For this review, take the finished solid that the model builds, in its own axes (mm). A direction names the side the tool comes from. Coordinates: 2 decimals unless noted, no trailing zeros. Loops run counter-clockwise (first coordinate to the right, second up) from the corner with the lowest first, then second, coordinate; pieces in that order, holes last. Notation, with made-up numbers: M -32,48 L 26,48 A16 ccw 26,73 Z; hole C -25,21.25 d8. An arc over 180 degrees is marked long. Use one line per item in the form item = value.
```python
from build123d import *

# Parameters (mm, degrees)
SKETCH1_R             = 25.1
BOSS_EXTRUDE1_DEPTH   = 6
FILLET1_R             = 4
FILLET2_R             = 2
CHAMFER1_SIZE         = 1
M5_TAPPED_HOLE2_D     = 4.2
M5_TAPPED_HOLE1_D     = 4.2
M5_TAPPED_HOLE1_DEPTH = 14
M5_TAPPED_HOLE1_TIP   = 1.2618073
CHAMFER2_SIZE         = 1


with BuildPart() as part:
    # Sketch1 → Boss-Extrude1 (new, symmetric)
    with BuildSketch(Plane(origin=(0, 0, 0), x_dir=(0, 0, -1), z_dir=(1, 0, 0))):
        Polygon((-45, 0), (45, 0), (45, 12), (30, 12), (30, 72), (-30, 72), (-30, 12), (-45, 12), align=None)
        with Locations((0, 42)):
            Circle(SKETCH1_R, mode=Mode.SUBTRACT)
    extrude(amount=BOSS_EXTRUDE1_DEPTH, both=True)

    # Fillet1
    fillet1_edges = [part.edges().sort_by_distance(p)[0] for p in [
        (0, 72, 30),
        (0, 72, -30),
    ]]
    fillet(fillet1_edges, radius=FILLET1_R)

    # Fillet2
    fillet2_edges = [part.edges().sort_by_distance(p)[0] for p in [
        (0, 12, 30),
        (0, 12, -30),
    ]]
    fillet(fillet2_edges, radius=FILLET2_R)

    # Chamfer1
    chamfer1_edges = [part.edges().sort_by_distance(p)[0] for p in [
        (0, 12, 45),
        (0, 12, -45),
    ]]
    chamfer(chamfer1_edges, length=CHAMFER1_SIZE)

    # M5 Tapped Hole2 (through all)
    with Locations(Plane(origin=(0, 12, 0), x_dir=(1, 0, 0), z_dir=(0, 1, 0))):
        with Locations((0, -37.5), (0, 37.5)):
            Hole(M5_TAPPED_HOLE2_D / 2)

    # M5 Tapped Hole1
    with Locations(Plane(origin=(6, 0, 0), x_dir=(0, 0, -1), z_dir=(1, 0, 0))):
        with Locations((-24.748737342, 66.748737342), (24.748737342, 66.748737342), (24.748737342, 17.251262658), (-24.748737342, 17.251262658)):
            Hole(M5_TAPPED_HOLE1_D / 2, depth=M5_TAPPED_HOLE1_DEPTH)
            with Locations((0, 0, -(M5_TAPPED_HOLE1_DEPTH + M5_TAPPED_HOLE1_TIP / 2))):  # 118° drill point
                Cone(0, M5_TAPPED_HOLE1_D / 2, M5_TAPPED_HOLE1_TIP, mode=Mode.SUBTRACT)

    # Chamfer2
    chamfer2_edges = [part.edges().sort_by_distance(p)[0] for p in [
        (-6, 42, 25.1),
        (6, 42, 25.1),
    ]]
    chamfer(chamfer2_edges, length=CHAMFER2_SIZE)


solid = part.part
```
1. Tool access review of faces 1 (the face through (-0.08, 64.7, 24.29)), 2 (the face through (1.42, 12, 39.25)), 3 (the face through (1.4, 12, -39.4)): name each direction out of +Z, -Z, +X, -X, +Y, -Y from which nothing blocks a thin tool from reaching the whole face with its end or side.
Computed values:
face_1 = +X, -X
face_2 = +Z, +X, -X, +Y
face_3 = -Z, +X, -X, +Y
2. Consider section B-B on y = 42. Write out the cut boundary in (x, z), plus the area to 3 significant figures.
Computed values:
outline = M -6,-30 L 6,-30 L 6,-26.1 L 5,-25.1 L -5,-25.1 L -6,-26.1 Z; M -6,26.1 L -5,25.1 L 5,25.1 L 6,26.1 L 6,30 L -6,30 Z
area = 116 mm2
3. For pin 1 Ø4 at (x, y) = (3.5, 53.5) entering from +Z; pin 2 Ø3 at (x, y) = (-4.5, 24.5) entering from -Z; pin 3 Ø4 at (y, z) = (66.75, -24.75) entering from -X; pin 4 Ø5 at (x, z) = (0, 37.5) entering from +Y, all flat-tipped, find the tip position at first contact; note any pin that passes through.
Computed values:
pin_1 = 30
pin_2 = -30
pin_3 = through
pin_4 = 12
4. Consider section A-A on z = 0. Write out the cut boundary in (x, y), plus the area to 3 significant figures.
Computed values:
outline = M -6,0 L 6,0 L 6,15.9 L 5,16.9 L -5,16.9 L -6,15.9 Z; M -6,68.1 L -5,67.1 L 5,67.1 L 6,68.1 L 6,72 L -6,72 Z
area = 260 mm2
5. Consider section C-C on x = -1. Write out the cut boundary in (y, z).
Computed values:
outline = M 0,-45 L 11,-45 L 12,-44 L 12,-39.35 L 0,-39.35 Z; M 0,-35.65 L 12,-35.65 L 12,-32 A2 cw 14,-30 L 68,-30 A4 ccw 72,-26 L 72,26 A4 ccw 68,30 L 14,30 A2 cw 12,32 L 12,35.65 L 0,35.65 Z; M 0,39.35 L 12,39.35 L 12,44 L 11,45 L 0,45 Z; hole C 17.25,-24.75 d4.2; hole C 17.25,24.75 d4.2; hole C 42,0 d50.2; hole C 66.75,-24.75 d4.2; hole C 66.75,24.75 d4.2
6. Consider section D-D on z = -37.5. Write out the cut boundary in (x, y).
Computed values:
outline = M -6,0 L -2.1,0 L -2.1,12 L -6,12 Z; M 2.1,0 L 6,0 L 6,12 L 2.1,12 Z
7. Wall thickness on line 1 along Z through (x, y) = (0, 4); line 2 along Z through (x, y) = (-2.5, 41.5); line 3 along Y through (x, z) = (-0.75, 26.5): over which ranges is each line inside the solid? List them lowest first. Write a range as from..to.
Computed values:
line_1 = -45..-39.6, -35.4..35.4, 39.6..45
line_2 = -30..-25.1, 25.1..30
line_3 = 0..16.09, 18.41..65.59, 67.91..71.97
8. Draft analysis for pull direction X (two halves, no side actions). For faces 4 (the face through (-6, 21, -19)), 5 (the face through (0.46, 5.92, 39.55)), 6 (the face through (0, 41, 30)), state which applies: +X half, -X half, draft (parallel to the pull), parting line (faces both ways), or undercut.
Computed values:
face_4 = -X half
face_5 = undercut
face_6 = draft
